Source: CAD feature listing. Evaluate the final solid. Frame: model axes, mm. A direction names the side the tool comes from. Give positions to 0.01 mm unless a question says otherwise; leave off trailing zeros. Write each loop counter-clockwise with the first axis right and the second up, starting at its lowest first coordinate (ties: lowest second). Pieces come first, ordered by that corner, then holes. Notation, with made-up numbers: (88, 66.5) -> (103, 66.5) arc R31 cw to (103, 104.5) -> close; hole circle Ø8 at (47, 56). An arc over 180 degrees is marked (long way). Write item = value, one per line.
from build123d import *

# Parameters (mm, degrees)
SKETCH_1_W          = 80
SKETCH_1_H          = 60
SKETCH_1_W_2        = 74
SKETCH_1_H_2        = 54
EXTRUDE_1_DEPTH     = 740
SKETCH_3_W          = 80
SKETCH_3_H          = 60
CUT_EXTRUDE_1_DEPTH = 25
SKETCH_4_W          = 80
SKETCH_4_H          = 60
CUT_EXTRUDE_2_DEPTH = 25
SKETCH_5_W          = 80
SKETCH_5_H          = 60
SKETCH_5_W_2        = 74
SKETCH_5_H_2        = 54
EXTRUDE_2_DEPTH     = 25
SKETCH_6_W          = 80
SKETCH_6_H          = 60
SKETCH_6_W_2        = 74
SKETCH_6_H_2        = 54
EXTRUDE_3_DEPTH     = 25
SKETCH_7_W          = 45
SKETCH_7_H          = 5
CUT_EXTRUDE_3_DEPTH = 80
EXTRUDE_4_DEPTH     = 45
EXTRUDE_5_DEPTH     = 45
SKETCH_10_W         = 74
SKETCH_10_H         = 54
SKETCH_10_W_2       = 70
SKETCH_10_H_2       = 50
EXTRUDE_6_DEPTH     = 740


with BuildPart() as part:
    # 草图1 → 凸台-拉伸1 (new body)
    with BuildSketch(Plane.XY):
        with Locations((40, -30)):
            Rectangle(SKETCH_1_W, SKETCH_1_H)
        with Locations((40, -30)):
            Rectangle(SKETCH_1_W_2, SKETCH_1_H_2, mode=Mode.SUBTRACT)
    extrude(amount=EXTRUDE_1_DEPTH)

    # 草图3 → 切除-拉伸1 (cut)
    with BuildSketch(Plane.XY.offset(740)):
        with Locations((40, -30)):
            Rectangle(SKETCH_3_W, SKETCH_3_H)
    extrude(amount=-CUT_EXTRUDE_1_DEPTH, mode=Mode.SUBTRACT)

    # 草图4 → 切除-拉伸2 (cut)
    with BuildSketch(Plane(origin=(0, 0, 0), x_dir=(-1, 0, 0), z_dir=(0, 0, -1))):
        with Locations((-40, -30)):
            Rectangle(SKETCH_4_W, SKETCH_4_H)
    extrude(amount=-CUT_EXTRUDE_2_DEPTH, mode=Mode.SUBTRACT)

    # 草图5 → 凸台-拉伸2 (add)
    with BuildSketch(Plane.XY.offset(715)):
        with Locations((40, -30)):
            Rectangle(SKETCH_5_W, SKETCH_5_H)
        with Locations((40, -30)):
            Rectangle(SKETCH_5_W_2, SKETCH_5_H_2, mode=Mode.SUBTRACT)
    extrude(amount=EXTRUDE_2_DEPTH)

    # 草图6 → 凸台-拉伸3 (add)
    with BuildSketch(Plane(origin=(0, 0, 25), x_dir=(-1, 0, 0), z_dir=(0, 0, -1))):
        with Locations((-40, -30)):
            Rectangle(SKETCH_6_W, SKETCH_6_H)
        with Locations((-40, -30)):
            Rectangle(SKETCH_6_W_2, SKETCH_6_H_2, mode=Mode.SUBTRACT)
    extrude(amount=EXTRUDE_3_DEPTH)

    # 草图7 → 切除-拉伸3 (cut)
    with BuildSketch(Plane(origin=(80, 0, 0), x_dir=(0, 0, -1), z_dir=(1, 0, 0))):
        with Locations((-717.5, -57.5)):
            Rectangle(SKETCH_7_W, SKETCH_7_H)
        with Locations((-22.5, -57.5)):
            Rectangle(SKETCH_7_W, SKETCH_7_H)
    extrude(amount=-CUT_EXTRUDE_3_DEPTH, mode=Mode.SUBTRACT)

    # 草图8 → 凸台-拉伸4 (add)
    with BuildSketch(Plane(origin=(0, 0, 45), x_dir=(-1, 0, 0), z_dir=(0, 0, -1))):
        Polygon((-3, -55), (-3, -57), (-77, -57), (-77, -55), (-80, -55), (-80, -60), (0, -60), (0, -55), align=None)
    extrude(amount=EXTRUDE_4_DEPTH)

    # 草图9 → 凸台-拉伸5 (add)
    with BuildSketch(Plane.XY.offset(695)):
        Polygon((3, -57), (3, -55), (0, -55), (0, -60), (80, -60), (80, -55), (77, -55), (77, -57), align=None)
    extrude(amount=EXTRUDE_5_DEPTH)

    # 草图10 → 凸台-拉伸6 (add)
    with BuildSketch(Plane(origin=(0, 0, 0), x_dir=(-1, 0, 0), z_dir=(0, 0, -1))):
        with Locations((-40, -30)):
            Rectangle(SKETCH_10_W, SKETCH_10_H)
        with Locations((-40, -30)):
            Rectangle(SKETCH_10_W_2, SKETCH_10_H_2, mode=Mode.SUBTRACT)
    extrude(amount=-EXTRUDE_6_DEPTH)


solid = part.part
(1) Section query B-B (z = 497). Return loops of the section in (x, y).
Values follow:
outline = (0, -60) -> (80, -60) -> (80, 0) -> (0, 0) -> close; hole (5, -55) -> (75, -55) -> (75, -5) -> (5, -5) -> close
(2) Pull-direction query (Y, two-part tool) for faces 1 (the face through (40, -3, 740)), 2 (the face through (41, 0, 375)), 3 (the face through (40, -5, 365)); classes: pulls with the +Y half, pulls with the -Y half, needs draft (parallel to the pull), parting line crosses it, or undercut.
Values follow:
face_1 = needs draft
face_2 = pulls with the +Y half
face_3 = undercut
(3) Section query A-A (x = 33.5). Return loops of the section in (y, z).
Values follow:
outline = (-60, 0) -> (-55, 0) -> (-55, 740) -> (-60, 740) -> close; (-5, 0) -> (0, 0) -> (0, 740) -> (-5, 740) -> close
(4) First-contact query: pin 1 (21 mm diameter, centred on x = 36, z = 376.5, fed in from +Y). Flat tip, straight axial feed; report the tip coordinate or a pass-through.
Values follow:
pin_1 = 0
(5) Access query for faces 4 (the face through (39, -60, 365)), 5 (the face through (5, -30, 365)). Directions: +Z, -Z, +X, -X, +Y, -Y. A direction counts if a zero-diameter tool reaches every point of the face in a straight line with its end or side. Return the directions, or none.
Values follow:
face_4 = +Z, -Z, +X, -X, -Y
face_5 = +Z, -Z
(6) Section query C-C (y = -27.5). Return loops of the section in (x, z), plus the area to 3 significant figures.
Values follow:
outline = (0, 0) -> (5, 0) -> (5, 740) -> (0, 740) -> close; (75, 0) -> (80, 0) -> (80, 740) -> (75, 740) -> close
area = 7,400 mm2
(7) Material intervals for line 1 (X direction, y = -54.5, z = 226); line 2 (Y direction, x = 54, z = 163), sorted ascending.
Values follow:
line_1 = 0 to 5, 75 to 80
line_2 = -60 to -55, -5 to 0
